For this review, use the dimensioned drawing (mm, ordinates from the lowest corner) and the shaded views. A direction names the side the tool comes from. Give positions to 0.01 mm unless a question says otherwise; leave off trailing zeros. Order: outer loops, then holes, each group sorted by start corner. A loop starts at its lowest first (then second) coordinate and runs counter-clockwise, first axis right, second up. Notation, with made-up numbers: (26.5, 18) -> (85.5, 18) arc R11 cw to (85.5, 37) -> close; hole circle Ø9 at (-23, 51). An arc over 180 degrees is marked (long way). Return JSON: item names as keys, results as strings.
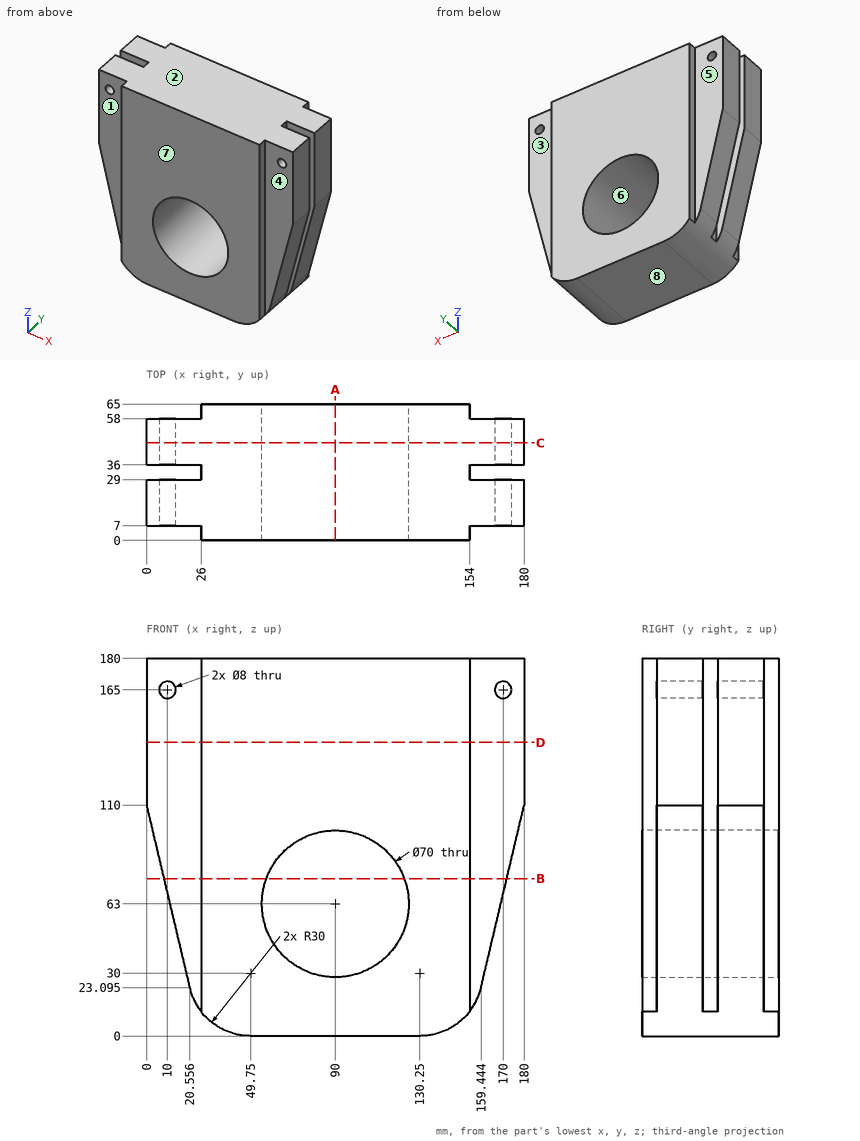
Item 1: Wall thickness on L1, parallel to Y at x = 17, z = 42; L2, parallel to Z at x = 131.5, y = 54; L3, parallel to X at y = 32.5, z = 161: over which ranges is each line inside the solid? List them lowest first. Write a range as [from, to].
Result set:
{"L1": "y = [7, 29], [36, 58]", "L2": "z = [0.03, 180]", "L3": "x = [26, 154]"}
Item 2: Mouldability with a two-part tool opening along Z and no side actions: class the marked faces 6, 7 and 8 as released by +Z, released by -Z, zero draft, split by the parting line, or undercut.
Result set:
{"face 6": "undercut", "face 7": "zero draft", "face 8": "released by -Z"}
Item 3: Machinability: for the marked faces 1, 2, 3, 4 and 5, which of the approach directions +Z, -Z, +X, -X, +Y, -Y give a long, thin tool a straight path to every point of the face, cutting with its end or side? Answer none if there is none.
Result set:
{"face 1": "+Z, -Z, -X, -Y", "face 2": "+Z, +X, -X, +Y, -Y", "face 3": "+Z, -Z, +X, +Y", "face 4": "+Z, -Z, +X, -Y", "face 5": "+Z, -Z, -X, +Y"}
Item 4: Add section C-C (y = 46.5). Give the number of separate pieces and of enclosed holes in the cut face, plus the area to 3 significant figures.
Result set:
{"separate pieces": "1", "enclosed holes": "3", "area": "25,400 mm^2"}
Item 5: Add section B-B (z = 75). Give the boundary of the cut face in (x, y).
Result set:
{"outline": "(8.28, 7) -> (26, 7) -> (26, 0) -> (57.12, 0) -> (57.12, 65) -> (26, 65) -> (26, 58) -> (8.28, 58) -> (8.28, 36) -> (26, 36) -> (26, 29) -> (8.28, 29) -> close; (122.88, 0) -> (154, 0) -> (154, 7) -> (171.72, 7) -> (171.72, 29) -> (154, 29) -> (154, 36) -> (171.72, 36) -> (171.72, 58) -> (154, 58) -> (154, 65) -> (122.88, 65) -> close"}
Item 6: Add section D-D (z = 140). Give the boundary of the cut face in (x, y), plus the area to 3 significant figures.
Result set:
{"outline": "(0, 7) -> (26, 7) -> (26, 0) -> (154, 0) -> (154, 7) -> (180, 7) -> (180, 29) -> (154, 29) -> (154, 36) -> (180, 36) -> (180, 58) -> (154, 58) -> (154, 65) -> (26, 65) -> (26, 58) -> (0, 58) -> (0, 36) -> (26, 36) -> (26, 29) -> (0, 29) -> close", "area": "10,600 mm^2"}
Item 7: For pin 1 (3.5 mm diameter, centred on y = 33.5, z = 62.5, fed in from +X); pin 2 (5.5 mm diameter, centred on y = 60.5, z = 76, fed in from +X); pin 3 (10.5 mm diameter, centred on x = 170, z = 165, fed in from +Y), all flat-tipped, find the tip position at first contact; note any pin that passes through.
Result set:
{"pin 1": "stops at x = 154", "pin 2": "stops at x = 172.23", "pin 3": "stops at y = 58"}
Item 8: Add section A-A (x = 90). Give the boundary of the cut face in (y, z).
Result set:
{"outline": "(0, 0) -> (65, 0) -> (65, 28) -> (0, 28) -> close; (0, 98) -> (65, 98) -> (65, 180) -> (0, 180) -> close"}
